from build123d import *

# Parameters (mm, degrees)
SKETCH1_W                                            = 800
SKETCH1_H                                            = 600
BOSS_EXTRUDE1_DEPTH                                  = 80
CHAMFER1_SIZE                                        = 5
CBORE_FOR_M16_HEX_SOCKET_HEAD_CAP_SCREW1_D           = 17.5
CBORE_FOR_M16_HEX_SOCKET_HEAD_CAP_SCREW1_CBORE_D     = 26
CBORE_FOR_M16_HEX_SOCKET_HEAD_CAP_SCREW1_CBORE_DEPTH = 16.6
SKETCH4_R                                            = 56
CUT_EXTRUDE1_DEPTH                                   = 40
CHAMFER2_SIZE                                        = 5
SKETCH6_R                                            = 45
SKETCH6_R_2                                          = 25
BOSS_EXTRUDE2_DEPTH                                  = 60
CBORE_FOR_M16_HEX_SOCKET_HEAD_CAP_SCREW2_D           = 17.5
CBORE_FOR_M16_HEX_SOCKET_HEAD_CAP_SCREW2_CBORE_D     = 26
CBORE_FOR_M16_HEX_SOCKET_HEAD_CAP_SCREW2_CBORE_DEPTH = 16.6
SKETCH10_R                                           = 8
CUT_EXTRUDE2_DEPTH                                   = 507.359556047
CIRPATTERN1_COUNT                                    = 12


with BuildPart() as part:
    # Sketch1 → Boss-Extrude1 (new body)
    with BuildSketch(Plane(origin=(0, 0, 0), x_dir=(1, 0, 0), z_dir=(0, 1, 0))):
        Rectangle(SKETCH1_W, SKETCH1_H)
    extrude(amount=BOSS_EXTRUDE1_DEPTH)

    # Chamfer1
    chamfer1_edges = [part.edges().sort_by_distance(p)[0] for p in [
        (400, 40, 300),
        (-400, 40, 300),
        (-400, 40, -300),
        (400, 40, -300),
    ]]
    chamfer(chamfer1_edges, length=CHAMFER1_SIZE)

    # CBORE for M16 Hex Socket Head Cap Screw1 (through all)
    with Locations(Plane(origin=(0, 80, 0), x_dir=(1, 0, 0), z_dir=(0, 1, 0))):
        with Locations((2.405406629, 39.927609732), (35.781027655, 17.880661619), (33.375621026, -22.046948113), (-2.405406629, -39.927609732), (-35.781027655, -17.880661619), (-33.375621026, 22.046948113)):
            CounterBoreHole(CBORE_FOR_M16_HEX_SOCKET_HEAD_CAP_SCREW1_D / 2, CBORE_FOR_M16_HEX_SOCKET_HEAD_CAP_SCREW1_CBORE_D / 2, CBORE_FOR_M16_HEX_SOCKET_HEAD_CAP_SCREW1_CBORE_DEPTH)

    # Sketch4 → Cut-Extrude1 (cut)
    with BuildSketch(Plane.XZ):
        with Locations(Location((0, 0, 0), (0, 0, 270))):
            Circle(SKETCH4_R)
    extrude(amount=-CUT_EXTRUDE1_DEPTH, mode=Mode.SUBTRACT)

    # Chamfer2
    chamfer2_edges = [part.edges().sort_by_distance(p)[0] for p in [
        (0, 0, 56),
    ]]
    chamfer(chamfer2_edges, length=CHAMFER2_SIZE)

    # Sketch6 → Boss-Extrude2 (add)
    # profile 1 of 4: a face of its own
    with BuildSketch(Plane.XZ):
        with Locations(Location((-325, 225, 0), (0, 0, 90))):
            Circle(SKETCH6_R)
        with Locations(Location((-325, 225, 0), (0, 0, 270))):
            Circle(SKETCH6_R_2, mode=Mode.SUBTRACT)
    # profile 2 of 4: a face of its own
    with BuildSketch(Plane.XZ):
        with Locations(Location((325, 225, 0), (0, 0, 90))):
            Circle(SKETCH6_R)
        with Locations(Location((325, 225, 0), (0, 0, 270))):
            Circle(SKETCH6_R_2, mode=Mode.SUBTRACT)
    # profile 3 of 4: a face of its own
    with BuildSketch(Plane.XZ):
        with Locations(Location((-325, -225, 0), (0, 0, 90))):
            Circle(SKETCH6_R)
        with Locations(Location((-325, -225, 0), (0, 0, 270))):
            Circle(SKETCH6_R_2, mode=Mode.SUBTRACT)
    # profile 4 of 4: a face of its own
    with BuildSketch(Plane.XZ):
        with Locations(Location((325, -225, 0), (0, 0, 90))):
            Circle(SKETCH6_R)
        with Locations(Location((325, -225, 0), (0, 0, 270))):
            Circle(SKETCH6_R_2, mode=Mode.SUBTRACT)
    extrude(amount=BOSS_EXTRUDE2_DEPTH)

    # CBORE for M16 Hex Socket Head Cap Screw2 (through all)
    with Locations(Plane(origin=(0, 80, 0), x_dir=(1, 0, 0), z_dir=(0, 1, 0))):
        with Locations((-325, -225), (-325, 225), (325, 225), (325, -225)):
            CounterBoreHole(CBORE_FOR_M16_HEX_SOCKET_HEAD_CAP_SCREW2_D / 2, CBORE_FOR_M16_HEX_SOCKET_HEAD_CAP_SCREW2_CBORE_D / 2, CBORE_FOR_M16_HEX_SOCKET_HEAD_CAP_SCREW2_CBORE_DEPTH)

    # Sketch10 → Cut-Extrude2 (cut, through all)
    with BuildSketch(Plane.XZ):
        with Locations(Location((0, 200, 0), (0, 0, 270))):
            Circle(SKETCH10_R)
    cut_extrude2 = extrude(amount=-CUT_EXTRUDE2_DEPTH, mode=Mode.SUBTRACT)

    # CirPattern1: Cut-Extrude2 ×12 about axis
    cirpattern1_axis = Axis((0, 0, 0), (0, 1, 0))
    for i in range(1, CIRPATTERN1_COUNT):
        add(cut_extrude2.rotate(cirpattern1_axis, i * 360 / CIRPATTERN1_COUNT), mode=Mode.SUBTRACT)


solid = part.part
For this review, take the finished solid that the model builds, in its own axes (mm). A direction names the side the tool comes from. Round coordinates to 2 decimals unless told otherwise and drop trailing zeros. Write each loop counter-clockwise with the first axis right and the second up, starting at its lowest first coordinate (ties: lowest second). Pieces come first, ordered by that corner, then holes. Notation, with made-up numbers: (-34.5, -34) - (19.5, -34) arc R17 ccw to (19.5, -30) - close; hole circle Ø7 at (-40, 52). An arc over 180 degrees is marked (long way). Write item = value, one per line. Start each with the question number.
1. Wall thickness on L1, parallel to Z at x = -325, y = 35; L2, parallel to X at y = 67, z = -40; L3, parallel to X at y = 18.5, z = -225: over which ranges is each line inside the solid? List them lowest first.
2. For pin 1 Ø3 at (x, z) = (-249, -206) entering from -Y; pin 2 Ø8 at (x, z) = (-4, -35) entering from +Y; pin 3 Ø16 at (x, z) = (33.38, 22.05) entering from +Y, all flat-tipped, find the tip position at first contact; note any pin that passes through.
3. Consider section A-A on y = -32.5. State the section outline as (x, z) points.
4. Consider section B-B on z = 225. Give the number of separate pieces and of enclosed holes in the cut face, plus the area to 3 significant figures.
5. For faces 1 (the face through (-329.7, 31.26, -232.38)), 2 (the face through (1, 40, 1)), 3 (the face through (0.713, 71.816, -52.817)), list the 3-axis set-ups (+Z, -Z, +X, -X, +Y, -Y) from which the entire face can be reached by the end or side of a thin tool; tool diameter is ignored.
6. Draft analysis for pull direction Z (two halves, no side actions). For faces 4 (the face through (-400, 39, 4)), 5 (the face through (-6, 39, 300)), 6 (the face through (-92.008, 39.44, 172.853)), 7 (the face through (-54.67, 22.26, 12.14)), state which applies: released by +Z, released by -Z, zero draft, split by the parting line, or undercut.
7. Consider section D-D on z = -156. State the section outline as (x, y) points.
Evaluation:
q1.L1 = -300 to -233.75, -216.25 to 216.25, 233.75 to 300
q1.L2 = -400 to -10.59, 15.41 to 400
q1.L3 = -400 to -333.75, -316.25 to 316.25, 333.75 to 400
q2.pin_1 = 0
q2.pin_2 = 63.4
q2.pin_3 = through
q3.outline = circle Ø90 at (-325, -225); circle Ø90 at (-325, 225); circle Ø90 at (325, -225); circle Ø90 at (325, 225); hole circle Ø50 at (-325, -225); hole circle Ø50 at (-325, 225); hole circle Ø50 at (325, -225); hole circle Ø50 at (325, 225)
q4.separate_pieces = 3
q4.enclosed_holes = 0
q4.area = 65,700 mm2
q5.face_1 = +Y, -Y
q5.face_2 = -Y
q5.face_3 = +Y
q6.face_4 = zero draft
q6.face_5 = released by +Z
q6.face_6 = undercut
q6.face_7 = undercut
q7.outline = (-400, 0) - (400, 0) - (400, 80) - (-400, 80) - close
